Verification items for this drawing (mm, ordinates from the low corner). A direction names the side the tool comes from. Give positions to 0.01 mm unless a question says otherwise; leave off trailing zeros. Loops run counter-clockwise (first coordinate to the right, second up) from the corner with the lowest first, then second, coordinate; pieces in that order, holes last. Notation, with made-up numbers: (7.5, 79.5) - (40.5, 79.5) arc R22 ccw to (40.5, 117.5) - close; hole circle Ø1 at (-7.75, -26.5). An arc over 180 degrees is marked (long way). One line per question, with ' | ' between items. Start each with the question number.
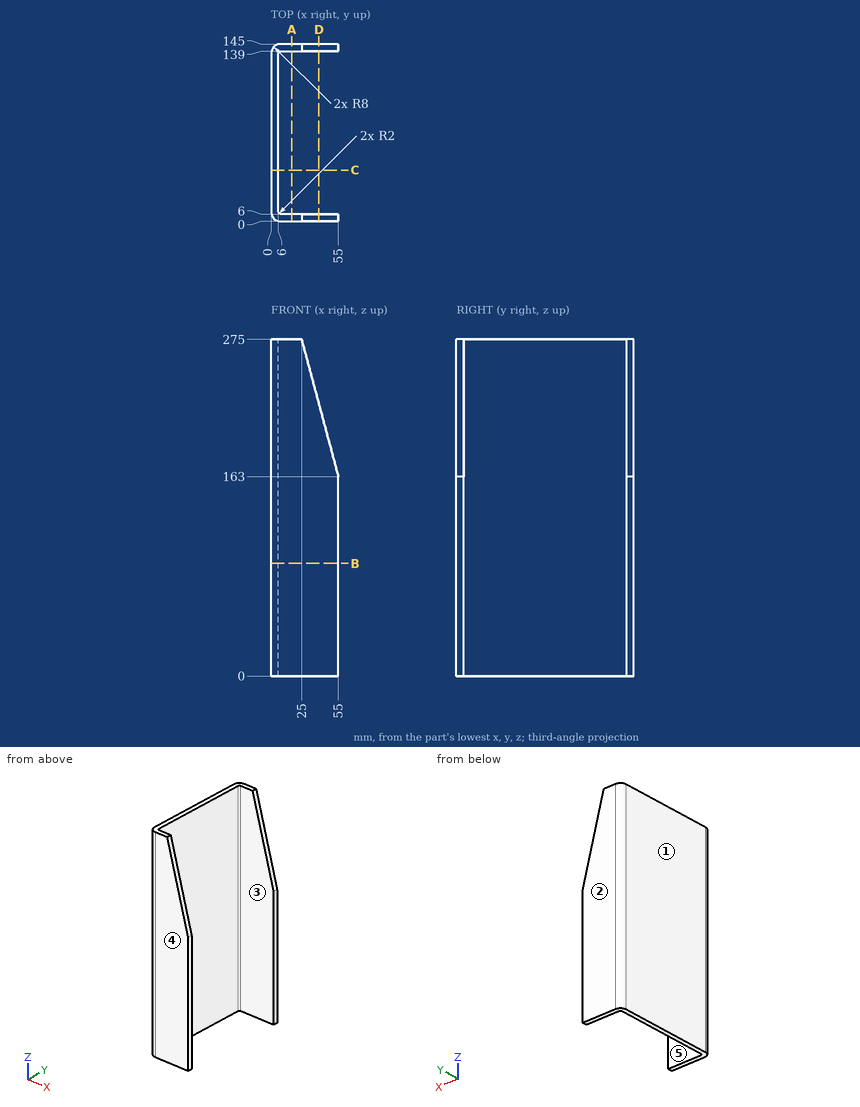
(1) Section check A-A, the plane x = 17. Record the boundary of the cut face in (y, z).
(2) Section check D-D, the plane x = 39. Record the boundary of the cut face in (y, z), and give its area (3 significant figures).
(3) Section check C-C, the plane y = 42. Record the boundary of the cut face in (x, z), and give its area (3 significant figures).
(4) Material ranges on line 1 (Y direction, x = 48, z = 177.5); line 2 (X direction, y = 23, z = 261); line 3 (Y direction, x = 3.5, z = 202), recorded low to high.
(5) Tool access check on the marked faces 4 and 5. Record the directions out of +Z, -Z, +X, -X, +Y, -Y that give a thin tool (end or side, any length) a straight path to the whole face; none if there is none.
(6) Mould release check, pull along Y, two halves, no side actions. Record for the marked faces 1, 2 and 3: pulls with the +Y half, pulls with the -Y half, needs draft (parallel to the pull), parting line crosses it, or undercut.
(7) Section check B-B, the plane z = 92. Record the boundary of the cut face in (x, y), and give its area (3 significant figures).
(8) Depth check by flat-ended pin: pin 1 Ø1.5 at (x, z) = (15.5, 103) entering from -Y; pin 2 Ø10 at (y, z) = (82, 176.5) entering from +X. Enter the tip coordinate at first touch or a pass-through.
Numbers:
1) outline: (0, 0) - (6, 0) - (6, 275) - (0, 275) - close; (139, 0) - (145, 0) - (145, 275) - (139, 275) - close
2) outline: (0, 0) - (6, 0) - (6, 222.73) - (0, 222.73) - close; (139, 0) - (145, 0) - (145, 222.73) - (139, 222.73) - close | area: 2,670 mm^2
3) outline: (0, 0) - (6, 0) - (6, 275) - (0, 275) - close | area: 1,650 mm^2
4) line 1: 0 to 6, 139 to 145 | line 2: 0 to 6 | line 3: 1.39 to 143.61
5) face 4: +Z, -Z, +X, -X, -Y | face 5: +Z, -Z, +X
6) face 1: needs draft | face 2: pulls with the +Y half | face 3: undercut
7) outline: (0, 8) arc R8 ccw to (8, 0) - (55, 0) - (55, 6) - (8, 6) arc R2 cw to (6, 8) - (6, 137) arc R2 cw to (8, 139) - (55, 139) - (55, 145) - (8, 145) arc R8 ccw to (0, 137) - close | area: 1,430 mm^2
8) pin 1: y = 0 | pin 2: x = 6
